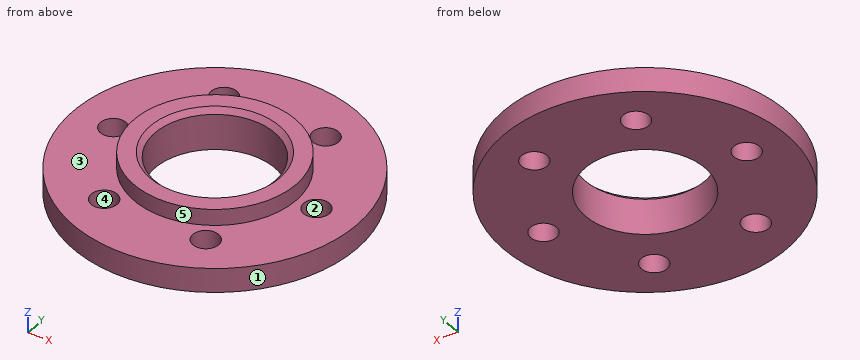
from build123d import *

# Parameters (mm, degrees)
SKETCH1_R                  = 50
BOSS_EXTRUDE1_DEPTH        = 10
SKETCH2_R                  = 87.5
BOSS_EXTRUDE2_DEPTH        = 15
CUT_EXTRUDE1_REACH         = 128.244
SKETCH3_R                  = 37
F_16_0_16_DIAMETER_HOLE1_D = 16
CHAMFER1_SIZE              = 3


with BuildPart() as part:
    # Sketch1 → Boss-Extrude1 (new body)
    with BuildSketch(Plane.XY):
        Circle(SKETCH1_R)
    extrude(amount=BOSS_EXTRUDE1_DEPTH)

    # Sketch2 → Boss-Extrude2 (add)
    with BuildSketch(Plane.XY):
        Circle(SKETCH2_R)
    extrude(amount=-BOSS_EXTRUDE2_DEPTH)

    # Sketch3 → Cut-Extrude1 (cut, up to next)
    with BuildSketch(Plane.XY.offset(10), mode=Mode.PRIVATE) as cut_extrude1_sk1:
        Circle(SKETCH3_R)
    cut_extrude1_tool1 = extrude(cut_extrude1_sk1.sketch, amount=-CUT_EXTRUDE1_REACH, mode=Mode.PRIVATE) & part.part
    add(cut_extrude1_tool1.solids().sort_by_distance((0, 0, 10))[0], mode=Mode.SUBTRACT)

    # Ø16.0 (16) Diameter Hole1 (through all)
    with Locations(Plane.XY):
        with Locations((62.5, 0), (31.25, -54.126587737), (-31.25, -54.126587737), (-62.5, 0), (-31.25, 54.126587737), (31.25, 54.126587737)):
            Hole(F_16_0_16_DIAMETER_HOLE1_D / 2)

    # Chamfer1
    chamfer1_edges = [part.edges().sort_by_distance(p)[0] for p in [
        (-37, 0, 10),
    ]]
    chamfer(chamfer1_edges, length=CHAMFER1_SIZE)


solid = part.part
Build history of the part. All positions in model axes, mm. Face numbers are marked on the shaded views. A direction names the side the tool comes from. Round coordinates to 2 decimals unless told otherwise and drop trailing zeros. Loops run counter-clockwise (first coordinate to the right, second up) from the corner with the lowest first, then second, coordinate; pieces in that order, holes last. Notation, with made-up numbers: (5.5, -12) -> (29.5, -12) arc R37 cw to (29.5, 27) -> close; hole circle Ø11 at (-20.5, 13). An arc over 180 degrees is marked (long way). Use CSV: the item, a comma, the result in double quotes. Start each with the question number.
Q1. Saw through at C-C on z = -9.5. Give the cut face in (x, y).
Q2. Mould opens along X. For the marked faces 1, 2 and 3 say: +X half, -X half, draft (parallel to the pull), parting line (faces both ways), or undercut.
Q3. Flat gauge pins, fed straight in: pin 1 Ø3 at (x, z) = (-3.5, -5) entering from +Y; pin 2 Ø1 at (x, y) = (27, -24.5) entering from +Z; pin 3 Ø12 at (x, z) = (67, -10) entering from -Y; pin 4 Ø10 at (x, z) = (40.5, 6) entering from +Y. Where does each tip first touch, or does it go through?
Q4. Drill centre lines: L1, parallel to X at y = -57, z = -6; L2, parallel to Y at x = 0, z = -2.5; L3, parallel to Y at x = 31.25, z = -2.75. Where is each one in solid material? Low to high.
Q5. Saw through at D-D on x = 66.5. Give the cut face in (y, z), and give its area (3 significant figures).
Q6. Saw through at B-B on x = 0. Give the cut face in (y, z).
Q7. Which spindle directions (+Z, -Z, +X, -X, +Y, -Y) get a long thin tool onto all of the face, cutting with end or side? Do the marked faces 4 and 5. Say none if no direction does.
Q8. Saw through at A-A on y = 0. Give the cut face in (x, z), and give its area (3 significant figures).
Solutions:
1,outline,"circle Ø175 at (0, 0); hole circle Ø16 at (-62.5, 0); hole circle Ø16 at (-31.25, -54.13); hole circle Ø16 at (-31.25, 54.13); hole circle Ø74 at (0, 0); hole circle Ø16 at (31.25, -54.13); hole circle Ø16 at (31.25, 54.13); hole circle Ø16 at (62.5, 0)"
2,face 1,"parting line"
2,face 2,"undercut"
2,face 3,"draft"
3,pin 1,"stops at y = 87.48"
3,pin 2,"passes through"
3,pin 3,"stops at y = -62.73"
3,pin 4,"stops at y = 35.21"
4,L1,"x = -66.39 to -38.72, -23.78 to 23.78, 38.72 to 66.39"
4,L2,"y = -87.5 to -37, 37 to 87.5"
4,L3,"y = -81.73 to -62.13, -46.13 to -19.81, 19.81 to 46.13, 62.13 to 81.73"
5,outline,"(-56.87, -15) -> (-6.93, -15) -> (-6.93, 0) -> (-56.87, 0) -> close; (6.93, -15) -> (56.87, -15) -> (56.87, 0) -> (6.93, 0) -> close"
5,area,"1,500 mm^2"
6,outline,"(-87.5, -15) -> (-37, -15) -> (-37, 7) -> (-40, 10) -> (-50, 10) -> (-50, 0) -> (-87.5, 0) -> close; (37, -15) -> (87.5, -15) -> (87.5, 0) -> (50, 0) -> (50, 10) -> (40, 10) -> (37, 7) -> close"
7,face 4,"+Z, -Z"
7,face 5,"+Z"
8,outline,"(-87.5, -15) -> (-70.5, -15) -> (-70.5, 0) -> (-87.5, 0) -> close; (-54.5, -15) -> (-37, -15) -> (-37, 7) -> (-40, 10) -> (-50, 10) -> (-50, 0) -> (-54.5, 0) -> close; (37, -15) -> (54.5, -15) -> (54.5, 0) -> (50, 0) -> (50, 10) -> (40, 10) -> (37, 7) -> close; (70.5, -15) -> (87.5, -15) -> (87.5, 0) -> (70.5, 0) -> close"
8,area,"1,290 mm^2"
